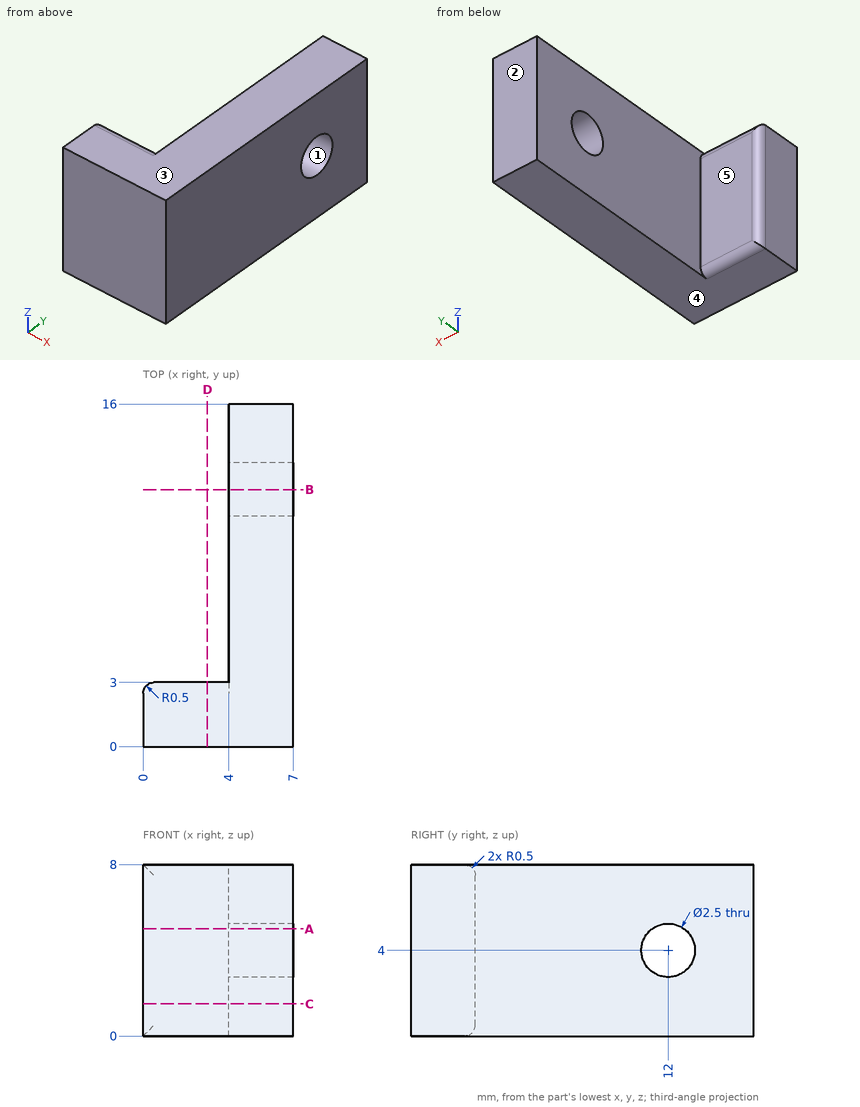
Study the drawing (mm; zero at the part's minimum x, y, z) and answer. A direction names the side the tool comes from. Round coordinates to 2 decimals unless told otherwise and drop trailing zeros. Write each loop counter-clockwise with the first axis right and the second up, starting at its lowest first coordinate (ties: lowest second). Pieces come first, ordered by that corner, then holes.
1) A cutting plane is placed at C-C on z = 1.5. Determine the outline of the cut face in (x, y), and give its area (3 significant figures).
2) Flat-ended cylindrical pins translate along their axes: P1, Ø1, axis at x = 2.5, y = 9.5, coming from the +Z side; P2, Ø1, axis at x = 1.5, z = 4, coming from the +Y side; P3, Ø2, axis at y = 10.5, z = 1.5, coming from the -X side; P4, Ø3, axis at y = 3.5, z = 2.5, coming from the -X side. Find the tip coordinate at first contact, or state that the pin passes through.
3) A cutting plane is placed at B-B on y = 12. Determine the outline of the cut face in (x, z).
4) Consider probe 1 along Y at (x, z) = (5.75, 4); probe 2 along X at (y, z) = (13.5, 1.5); probe 3 along Z at (x, y) = (5.5, 11.25). Determine where each line is inside the solid, lowest interval first.
5) A cutting plane is placed at A-A on z = 5. Determine the outline of the cut face in (x, y).
6) Determine the mould class of the marked faces 1, 2 and 3 for opening direction Y: pulls with the +Y half, pulls with the -Y half, needs draft (parallel to the pull), parting line crosses it, or undercut.
7) A cutting plane is placed at D-D on x = 3. Determine the outline of the cut face in (y, z).
8) Which of the six approach directions +Z, -Z, +X, -X, +Y, -Y give full straight-line access (tool end or side, diameter ignored) to the marked faces 4 and 5?
Entries:
1. outline: (0, 0) - (7, 0) - (7, 16) - (4, 16) - (4, 3) - (0.5, 3) arc R0.5 ccw to (0, 2.5) - close
1. area: 59.9 mm2
2. P1: passes through
2. P2: stops at y = 3
2. P3: stops at x = 4
2. P4: stops at x = 0
3. outline: (4, 0) - (7, 0) - (7, 2.75) - (4, 2.75) - close; (4, 5.25) - (7, 5.25) - (7, 8) - (4, 8) - close
4. probe 1: y = 0 to 10.75, 13.25 to 16
4. probe 2: x = 4 to 7
4. probe 3: z = 0 to 3, 5 to 8
5. outline: (0, 0) - (7, 0) - (7, 11.25) - (4, 11.25) - (4, 3) - (0.5, 3) arc R0.5 ccw to (0, 2.5) - close; (4, 12.75) - (7, 12.75) - (7, 16) - (4, 16) - close
6. face 1: undercut
6. face 2: pulls with the +Y half
6. face 3: needs draft
7. outline: (0, 0) - (2.5, 0) arc R0.5 ccw to (3, 0.5) - (3, 7.5) arc R0.5 ccw to (2.5, 8) - (0, 8) - close
8. face 4: -Z, +X, -X, +Y, -Y
8. face 5: +Z, -Z, -X, +Y
